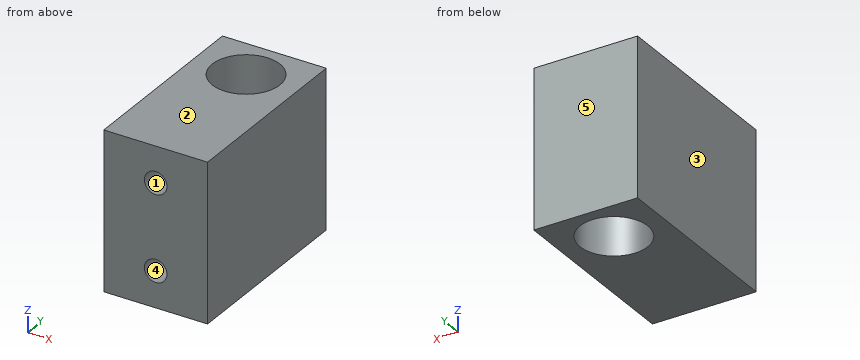
```python
from build123d import *

# Parameters (mm, degrees)
SKETCH_1_W          = 23
SKETCH_1_H          = 42
SKETCH_1_R          = 7.5
EXTRUDE_1_DEPTH     = 35
SKETCH_2_R          = 2.1
CUT_EXTRUDE_1_DEPTH = 11.5
SKETCH_3_R          = 2.5
CUT_EXTRUDE_2_DEPTH = 10


with BuildPart() as part:
    # 草图1 → 凸台-拉伸1 (new body)
    with BuildSketch(Plane.XY):
        with Locations((1.112903226, 1.756048387)):
            Rectangle(SKETCH_1_W, SKETCH_1_H)
        with Locations((1.112903226, 12.756048387)):
            Circle(SKETCH_1_R, mode=Mode.SUBTRACT)
    extrude(amount=EXTRUDE_1_DEPTH)

    # 草图2 → 切除-拉伸1 (cut)
    with BuildSketch(Plane.XZ.offset(19.243951613)):
        with Locations(Location((1.112903226, 27, 0), (0, 0, 270))):
            Circle(SKETCH_2_R)
        with Locations(Location((1.112903226, 8, 0), (0, 0, 270))):
            Circle(SKETCH_2_R)
    extrude(amount=-CUT_EXTRUDE_1_DEPTH, mode=Mode.SUBTRACT)

    # 草图3 → 切除-拉伸2 (cut)
    with BuildSketch(Plane.XZ.offset(19.243951613)):
        with Locations(Location((1.112903226, 27, 0), (0, 0, 270))):
            Circle(SKETCH_3_R)
        with Locations(Location((1.112903226, 8, 0), (0, 0, 270))):
            Circle(SKETCH_3_R)
    extrude(amount=-CUT_EXTRUDE_2_DEPTH, mode=Mode.SUBTRACT)


solid = part.part
```
Work out the finished part from the listing and answer in its coordinate system (mm). Face numbers are marked on the shaded views. A direction names the side the tool comes from. Coordinates: 2 decimals unless noted, no trailing zeros. Write each loop counter-clockwise with the first axis right and the second up, starting at its lowest first coordinate (ties: lowest second). Pieces come first, ordered by that corner, then holes. Notation, with made-up numbers: (-23, 78.5) - (-3, 78.5) arc R21 ccw to (-3, 103.5) - close; hole circle Ø4 at (34, 0). An arc over 180 degrees is marked (long way). Answer as a JSON object with one key per item and string values.
Q1. Which of the six approach directions +Z, -Z, +X, -X, +Y, -Y give full straight-line access (tool end or side, diameter ignored) to the marked faces 1 and 2?
Results list:
{"face 1": "-Y", "face 2": "+Z, +X, -X, +Y, -Y"}
Q2. Find section B-B (x = -5.75). Write down the section's boundary in (y, z).
Results list:
{"outline": "(-19.24, 0) - (9.73, 0) - (9.73, 35) - (-19.24, 35) - close; (15.78, 0) - (22.76, 0) - (22.76, 35) - (15.78, 35) - close"}
Q3. Consider L1, parallel to X at y = -8.1, z = 8; L2, parallel to X at y = -16.25, z = 27; L3, parallel to Y at x = 4.5, z = 26. Determine where each line is inside the solid, lowest interval first. Write a range as from..to.
Results list:
{"L1": "x = -10.39..-0.99, 3.21..12.61", "L2": "x = -10.39..-1.39, 3.61..12.61", "L3": "y = -19.24..6.06, 19.45..22.76"}
Q4. Find section C-C (z = 19.5). Write down the section's boundary in (x, y).
Results list:
{"outline": "(-10.39, -19.24) - (12.61, -19.24) - (12.61, 22.76) - (-10.39, 22.76) - close; hole circle Ø15 at (1.11, 12.76)"}
Q5. For a pull along X with two mould halves and no side action, classify the marked faces 3, 4 and 5 as pulls with the +X half, pulls with the -X half, needs draft (parallel to the pull), parting line crosses it, or undercut.
Results list:
{"face 3": "pulls with the -X half", "face 4": "undercut", "face 5": "needs draft"}
Q6. Given pin 1 Ø4 at (x, y) = (-4.5, -9) entering from -Z; pin 2 Ø4 at (x, z) = (1.5, 27) entering from -Y; pin 3 Ø9 at (x, y) = (1.11, 12.76) entering from +Z; pin 4 Ø1.5 at (x, z) = (1, 7.5) entering from -Y, each flat-ended and moving along its own axis, determine where each tip first touches the part or whether it passes through.
Results list:
{"pin 1": "stops at z = 0", "pin 2": "stops at y = -9.24", "pin 3": "passes through", "pin 4": "stops at y = -7.74"}
Q7. Find section D-D (y = -16). Write down the section's boundary in (x, z), plus the area to 3 significant figures.
Results list:
{"outline": "(-10.39, 0) - (12.61, 0) - (12.61, 35) - (-10.39, 35) - close; hole circle Ø5 at (1.11, 8); hole circle Ø5 at (1.11, 27)", "area": "766 mm^2"}
Q8. Find section A-A (y = 14.5). Write down the section's boundary in (x, z).
Results list:
{"outline": "(-10.39, 0) - (-6.18, 0) - (-6.18, 35) - (-10.39, 35) - close; (8.41, 0) - (12.61, 0) - (12.61, 35) - (8.41, 35) - close"}
